Check sheet for the drawn part. Datum: minimum x, y, z corner. Units: mm. Give positions to 0.01 mm unless a question says otherwise; leave off trailing zeros. Write each loop counter-clockwise with the first axis right and the second up, starting at its lowest first coordinate (ties: lowest second). Pieces come first, ordered by that corner, then holes. Notation, with made-up numbers: (-30.75, -6) -> (14.25, -6) arc R30 ccw to (14.25, 17) -> close; hole circle Ø10 at (20, 62.5). An arc over 180 degrees is marked (long way). Answer as CSV lines item,"result". Start each with the question number.
1) Sectioned sample at A-A on y = 115. Record the cut outline in (x, z).
2) Sectioned sample at B-B on z = 1.95. Record the cut outline in (x, y), and give its area (3 significant figures).
3) Material ranges on L1, parallel to Y at x = 115, z = 2.15; L2, parallel to X at y = 18, z = 3.5, recorded low to high.
4) Gauge pin test, flat end, axial feed: pin 1 Ø8 at (x, y) = (115, 15) entering from -Z. Record the tip position at first contact, or that the pin passes through.
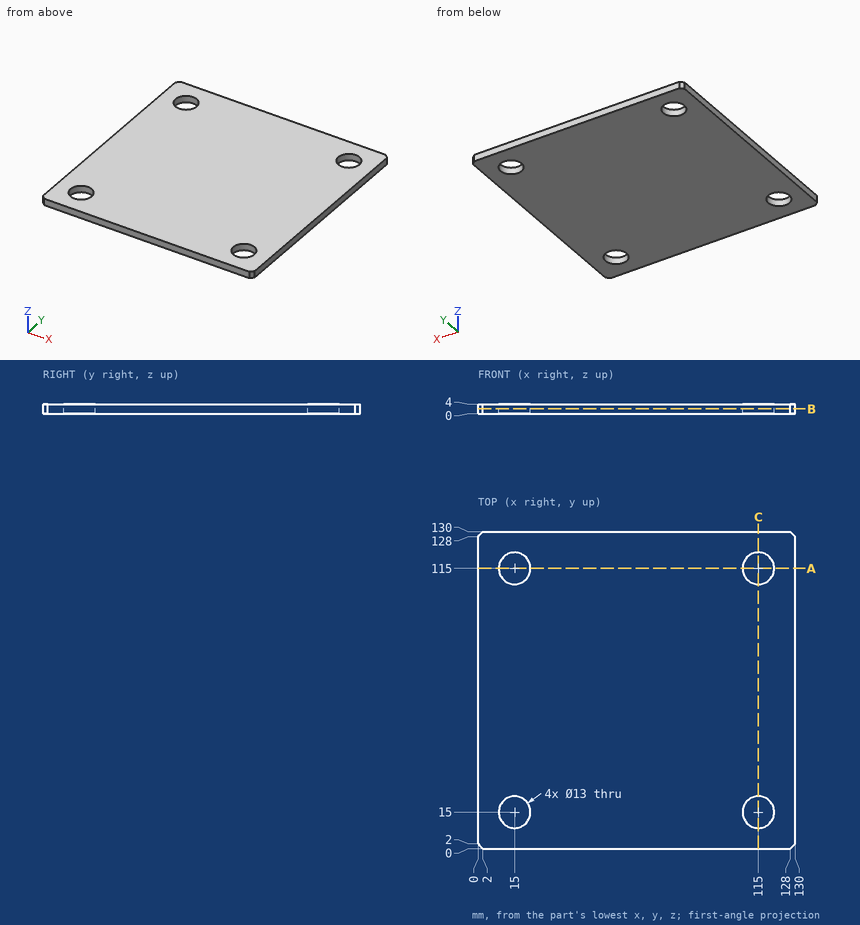
Ans:
1,outline,"(0, 0) -> (8.5, 0) -> (8.5, 4) -> (0, 4) -> close; (21.5, 0) -> (108.5, 0) -> (108.5, 4) -> (21.5, 4) -> close; (121.5, 0) -> (130, 0) -> (130, 4) -> (121.5, 4) -> close"
2,outline,"(0, 2) -> (2, 0) -> (128, 0) -> (130, 2) -> (130, 128) -> (128, 130) -> (2, 130) -> (0, 128) -> close; hole circle Ø13 at (15, 15); hole circle Ø13 at (15, 115); hole circle Ø13 at (115, 15); hole circle Ø13 at (115, 115)"
2,area,"16,400 mm²"
3,L1,"y = 0 to 8.5, 21.5 to 108.5, 121.5 to 130"
3,L2,"x = 0 to 9.23, 20.77 to 109.23, 120.77 to 130"
4,pin 1,"passes through"
